Print and shaded views of the part. All mm, measured from the part's lowest x, y and z. Round coordinates to 2 decimals unless told otherwise and drop trailing zeros. Loops run counter-clockwise (first coordinate to the right, second up) from the corner with the lowest first, then second, coordinate; pieces in that order, holes last. Notation, with made-up numbers: (-13.5, 22) -> (43.5, 22) arc R17 cw to (43.5, 41) -> close; hole circle Ø1 at (-6.5, 86.5). An arc over 180 degrees is marked (long way). Answer as CSV lines item,"result".
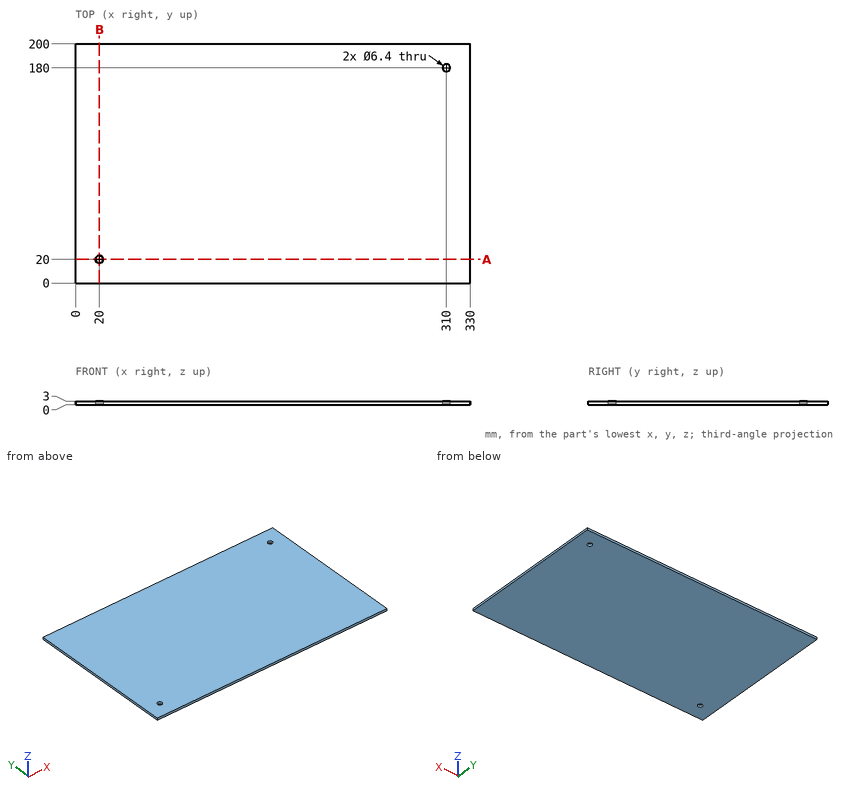
Q1. Saw through at A-A, the plane y = 20. Write the cut outline in (x, z).
Geometry results:
outline,"(0, 0) -> (16.8, 0) -> (16.8, 3) -> (0, 3) -> close; (23.2, 0) -> (330, 0) -> (330, 3) -> (23.2, 3) -> close"
Q2. Drop a flat-ended pin along its axis: P1, Ø6, axis at x = 20, y = 20, coming from the -Z side. Give the stop position or say it passes through.
Geometry results:
P1,"through"
Q3. Drill centre lines: line 1 along X through (y, z) = (180, 1.8); line 2 along Y through (x, z) = (310, 2.1); line 3 along X through (y, z) = (20, 1.55). Where is each one in solid material? Low to high.
Geometry results:
line 1,"0 to 306.8, 313.2 to 330"
line 2,"0 to 176.8, 183.2 to 200"
line 3,"0 to 16.8, 23.2 to 330"
Q4. Saw through at B-B, the plane x = 20. Write the cut outline in (y, z), then the cut area to 3 significant figures.
Geometry results:
outline,"(0, 0) -> (16.8, 0) -> (16.8, 3) -> (0, 3) -> close; (23.2, 0) -> (200, 0) -> (200, 3) -> (23.2, 3) -> close"
area,"581 mm2"
